Part print with two shaded views. Sizes in mm from the minimum x, y, z corner. A direction names the side the tool comes from. Give positions to 0.01 mm unless a question says otherwise; leave off trailing zeros. Loops run counter-clockwise (first coordinate to the right, second up) from the corner with the lowest first, then second, coordinate; pieces in that order, holes last. Notation, with made-up numbers: M -23,43.25 L 26,43.25 A11 ccw 26,50.25 Z; hole C -24,43.5 d7. An arc over 180 degrees is marked long. Answer as a JSON object with one key per item and string values. Group by question number.
1. Slice it at A-A (z = 3). List the corners of the cut face in (x, y).
2. Drill centre lines: line 1 along Y through (x, z) = (1.3, 3.5); line 2 along Y through (x, z) = (4.2, 3.6); line 3 along Z through (x, y) = (1.75, 35.5). Where is each one in solid material? Low to high. Write a range as [from, to].
3. Mould opens along Y. For the marked faces 3, 4 and 5 say: released by +Y, released by -Y, zero draft, split by the parting line, or undercut.
4. Drop a flat-ended pin along its axis: pin 1 Ø2 at (x, z) = (0.5, 1) entering from +Y. Give the stop position or say it passes through.
5. 3-axis set-ups, long thin cutter, end or side, ignore diameter. For the marked faces 1 and 2: which of +Z, -Z, +X, -X, +Y, -Y reach the whole face in a straight line?
6. Slice it at B-B (y = 8). List the corners of the cut face in (x, z), then the cut area to 3 significant figures.
7. Slice it at C-C (y = 31). List the corners of the cut face in (x, z).
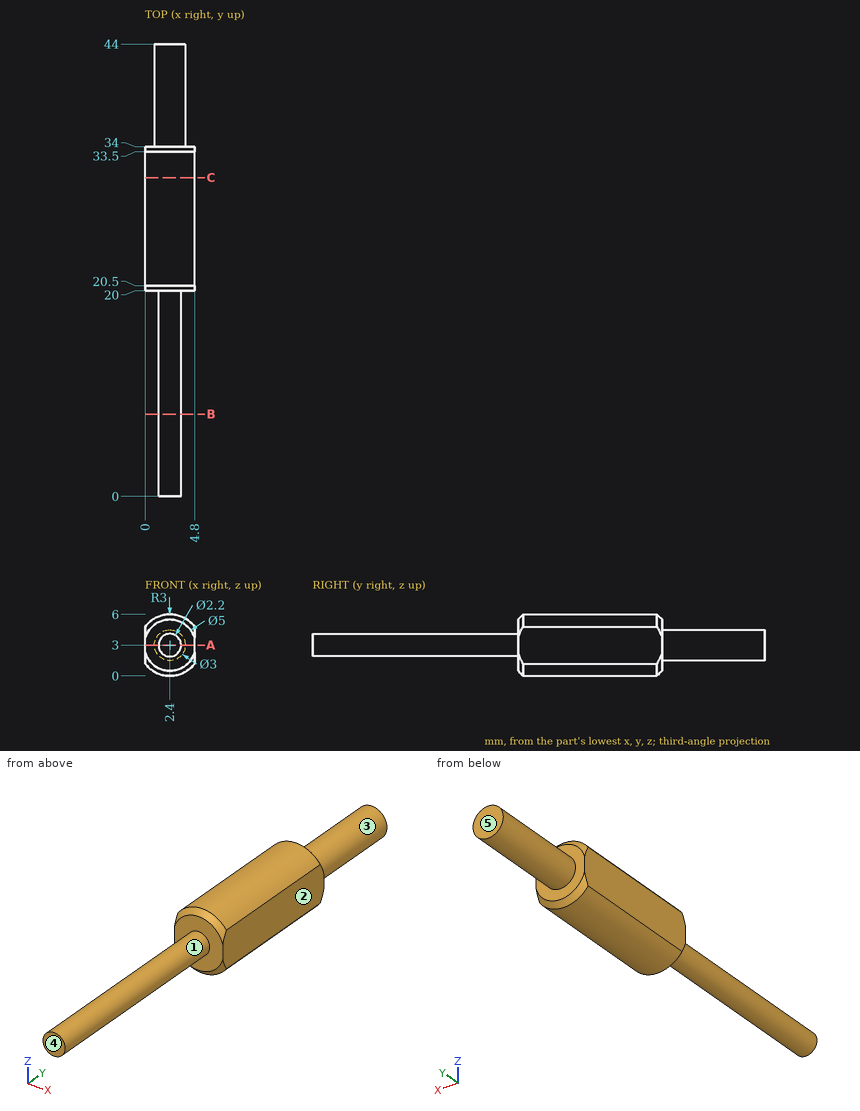
Established:
{
 "1": {"outline": "M 0,20 L 1.3,20 L 1.3,0 L 3.5,0 L 3.5,20 L 4.8,20 L 4.8,34 L 3.9,34 L 3.9,44 L 0.9,44 L 0.9,34 L 0,34 Z"},
 "2": {"line 1": "y = [20, 44]", "line 2": "y = [20, 34]", "line 3": "z = [1.65, 4.35]"},
 "3": {"face 3": "zero draft", "face 4": "released by -Y", "face 5": "released by +Y"},
 "4": {"pin 1": "stops at y = 34"},
 "5": {"face 1": "-Y", "face 2": "+Z, -Z, +X, +Y, -Y"},
 "6": {"outline": "C 2.4,3 d2.2", "area": "3.80 mm^2"},
 "7": {"outline": "M 0,1.2 A3 ccw 4.8,1.2 L 4.8,4.8 A3 ccw 0,4.8 Z"}
}
